For this review, take the finished solid that the model builds, in its own axes (mm). Coordinates: 2 decimals unless noted, no trailing zeros. Write each loop counter-clockwise with the first axis right and the second up, starting at its lowest first coordinate (ties: lowest second). Pieces come first, ordered by that corner, then holes. Notation, with made-up numbers: (74, 52) - (84, 52) arc R19 ccw to (84, 61) - close; hole circle Ø1 at (31.5, 74.5). An arc over 180 degrees is marked (long way). Write each question's results on one line, items separated by ' | '.
from build123d import *

# Parameters (mm, degrees)
SKETCH_1_W          = 40
SKETCH_1_H          = 40
EXTRUDE_1_DEPTH     = 18
SKETCH_2_R          = 8.2
CUT_EXTRUDE_1_DEPTH = 30


with BuildPart() as part:
    # 草图1 → 凸台-拉伸1 (new, symmetric)
    with BuildSketch(Plane.XY):
        Rectangle(SKETCH_1_W, SKETCH_1_H)
    extrude(amount=EXTRUDE_1_DEPTH, both=True)

    # 草图2 → 切除-拉伸1 (cut, symmetric)
    with BuildSketch(Plane.XY):
        Circle(SKETCH_2_R)
    extrude(amount=CUT_EXTRUDE_1_DEPTH, both=True, mode=Mode.SUBTRACT)


solid = part.part
Q1. Take a section at C-C on z = -5. State the section outline as (x, y) points.
Results found:
outline: (-20, -20) - (20, -20) - (20, 20) - (-20, 20) - close; hole circle Ø16.4 at (0, 0)
Q2. Mouldability with a two-part tool opening along Y and no side actions: class faces 1 (the face through (-1.07, 8.13, 0.25)), 2 (the face through (20, 0, 0)), 3 (the face through (0, 20, 0)) as pulls with the +Y half, pulls with the -Y half, needs draft (parallel to the pull), parting line crosses it, or undercut.
Results found:
face 1: undercut | face 2: needs draft | face 3: pulls with the +Y half
Q3. Take a section at A-A on x = 0. State the section outline as (y, z) points, plus the area to 3 significant figures.
Results found:
outline: (-20, -18) - (-8.2, -18) - (-8.2, 18) - (-20, 18) - close; (8.2, -18) - (20, -18) - (20, 18) - (8.2, 18) - close | area: 850 mm2
Q4. Wall thickness on line 1 along Y through (x, z) = (0, 8); line 2 along Y through (x, z) = (3, 8); line 3 along X through (y, z) = (-5.5, 6): over which ranges is each line inside the solid? List them lowest first. Write a range as from..to.
Results found:
line 1: -20..-8.2, 8.2..20 | line 2: -20..-7.63, 7.63..20 | line 3: -20..-6.08, 6.08..20
